Geometry check sheet. Reference: the model listing, model coordinates, mm. A direction names the side the tool comes from. Coordinates: 2 decimals unless noted, no trailing zeros. Write each loop counter-clockwise with the first axis right and the second up, starting at its lowest first coordinate (ties: lowest second). Pieces come first, ordered by that corner, then holes.
from build123d import *

# Parameters (mm, degrees)
SKETCH_1_W                  = 220
SKETCH_1_H                  = 12
EXTRUDE_1_DEPTH             = 60
HOLE_WIZARD_M6_1_D          = 5
HOLE_WIZARD_M6_1_DEPTH      = 13
HOLE_WIZARD_M6_1_TIP        = 1.502151548
HOLE_WIZARD_2_D             = 9
HOLE_WIZARD_2_CBORE_D       = 15
HOLE_WIZARD_2_CBORE_DEPTH   = 9
HOLE_WIZARD_2_2_D           = 6.6
HOLE_WIZARD_2_2_CBORE_D     = 11
HOLE_WIZARD_2_2_CBORE_DEPTH = 6.8
HOLE_WIZARD_M4_1_D          = 3.3
HOLE_WIZARD_M5_2_D          = 4.2
HOLE_WIZARD_M4_2_D          = 3.3
HOLE_WIZARD_M4_2_DEPTH      = 10.1
HOLE_WIZARD_M4_2_TIP        = 0.991420021


with BuildPart() as part:
    # 草图1 → 凸台-拉伸1 (new, symmetric)
    with BuildSketch(Plane.XY):
        Rectangle(SKETCH_1_W, SKETCH_1_H)
    extrude(amount=EXTRUDE_1_DEPTH, both=True)

    # M6 螺纹孔1
    with Locations(Plane(origin=(70, 0, -60), x_dir=(-1, 0, 0), z_dir=(0, 0, -1))):
        with Locations((0, 0), (70, 0), (140, 0)):
            Hole(HOLE_WIZARD_M6_1_D / 2, depth=HOLE_WIZARD_M6_1_DEPTH)
            with Locations((0, 0, -(HOLE_WIZARD_M6_1_DEPTH + HOLE_WIZARD_M6_1_TIP / 2))):  # 118° drill point
                Cone(0, HOLE_WIZARD_M6_1_D / 2, HOLE_WIZARD_M6_1_TIP, mode=Mode.SUBTRACT)

    # Hole Wizard 2 (through all)
    with Locations(Plane(origin=(-70, 6, -35), x_dir=(0, 0, 1), z_dir=(0, 1, 0))):
        with Locations((0, 0), (50, 0), (0, 140), (50, 140)):
            CounterBoreHole(HOLE_WIZARD_2_D / 2, HOLE_WIZARD_2_CBORE_D / 2, HOLE_WIZARD_2_CBORE_DEPTH)

    # Hole Wizard 2 2 (through all)
    with Locations(Plane(origin=(-28, -6, -27), x_dir=(0, 0, -1), z_dir=(0, -1, 0))):
        with Locations((0, 0), (0, 56), (-60, 56), (-60, 0)):
            CounterBoreHole(HOLE_WIZARD_2_2_D / 2, HOLE_WIZARD_2_2_CBORE_D / 2, HOLE_WIZARD_2_2_CBORE_DEPTH)

    # M4 螺纹孔1 (through all)
    with Locations(Plane(origin=(0, -6, 0), x_dir=(-1, 0, 0), z_dir=(0, -1, 0))):
        with Locations((26, -56), (60, -32)):
            Hole(HOLE_WIZARD_M4_1_D / 2)

    # M5 螺纹孔2 (through all)
    with Locations(Plane(origin=(0, -6, 0), x_dir=(-1, 0, 0), z_dir=(0, -1, 0))):
        with Locations((-56, -52), (-56, 47)):
            Hole(HOLE_WIZARD_M5_2_D / 2)

    # M4 螺纹孔2
    with Locations(Plane.XY.offset(60)):
        with Locations((-100, 0), (-80, 0)):
            Hole(HOLE_WIZARD_M4_2_D / 2, depth=HOLE_WIZARD_M4_2_DEPTH)
            with Locations((0, 0, -(HOLE_WIZARD_M4_2_DEPTH + HOLE_WIZARD_M4_2_TIP / 2))):  # 118° drill point
                Cone(0, HOLE_WIZARD_M4_2_D / 2, HOLE_WIZARD_M4_2_TIP, mode=Mode.SUBTRACT)


solid = part.part
1. Access from +Z, -Z, +X, -X, +Y, -Y to the whole of each face (thin tool, end or side, straight path). Record for faces 1 (the cylindrical face through (28.242, -2.648, 38.495)), 2 (the cylindrical face through (26.74, 3.44, -23.95)), 3 (the flat face through (70, -3, 20)).
Computed values:
face 1: -Y
face 2: +Y, -Y
face 3: +Y
2. Gauge pin test, flat ends, axial feed: pin 1 Ø5.5 at (x, z) = (29, 35) entering from -Y; pin 2 Ø3 at (x, y) = (0, 0) entering from -Z; pin 3 Ø4 at (x, z) = (-28, -27) entering from -Y; pin 4 Ø4.5 at (x, z) = (-67, 13) entering from +Y. Record the tip position at first contact, or that the pin passes through.
Computed values:
pin 1: stops at y = 0.8
pin 2: stops at z = -46.4
pin 3: passes through
pin 4: stops at y = -3
3. Draft check along Z on faces 4 (the cylindrical face through (-72, -1.5, -53.4)), 5 (the flat face through (-70, -3, 20)), 6 (the conical face through (0.094, -0.424, -45.759)). Enter one of: released by +Z, released by -Z, zero draft, split by the parting line, or undercut.
Computed values:
face 4: zero draft
face 5: undercut
face 6: released by -Z
4. Sectioned sample at A-A, the plane z = 15. Record the boundary of the cut face in (x, y).
Computed values:
outline: (-110, -6) - (-74.5, -6) - (-74.5, -3) - (-77.5, -3) - (-77.5, 6) - (-110, 6) - close; (-65.5, -6) - (65.5, -6) - (65.5, -3) - (62.5, -3) - (62.5, 6) - (-62.5, 6) - (-62.5, -3) - (-65.5, -3) - close; (74.5, -6) - (110, -6) - (110, 6) - (77.5, 6) - (77.5, -3) - (74.5, -3) - close
5. Thickness scan on line 1 along X through (y, z) = (4.85, -27); line 2 along Z through (x, y) = (-69.5, 5.75); line 3 along X through (y, z) = (1, -35). Record the ranges inside material, lowest first.
Computed values:
line 1: x = -110 to -31.3, -24.7 to 24.7, 31.3 to 110
line 2: z = -60 to -42.48, -27.52 to 7.52, 22.48 to 60
line 3: x = -110 to -77.5, -62.5 to 62.5, 77.5 to 110
